Part model, mm, in its own coordinate system. Coordinates: 2 decimals unless noted, no trailing zeros. Loops run counter-clockwise (first coordinate to the right, second up) from the corner with the lowest first, then second, coordinate; pieces in that order, holes last. Notation, with made-up numbers: M -21.5,4 L 5.5,4 A33 cw 5.5,36 Z; hole C 88.25,-14 d3. An arc over 180 degrees is marked long. Answer as a JSON object with one key per item and string values. Group by question number.
1. Saw through at B-B on x = 9. Write the cut outline in (y, z).
2. Saw through at A-A on y = 26. Write the cut outline in (x, z) (3 decimals).
3. Drop flat-ended pins along their axis: pin 1 Ø10.5 at (y, z) = (26, -20) entering from +X; pin 2 Ø8.5 at (y, z) = (-27, 20) entering from -X; pin 3 Ø2.5 at (x, z) = (5, 30) entering from +Y. Give the stop position or say it passes through.
4. Drill centre lines: L1, parallel to Z at x = 4.75, y = 26; L2, parallel to Y at x = 3.75, z = -20; L3, parallel to X at y = 26.25, z = 30. Where is each one in solid material? Low to high.
5. Saw through at C-C on z = 20. Write the cut outline in (x, y) (3 decimals), then the cut area to 3 significant figures.
6. Saw through at D-D on y = -27. Write the cut outline in (x, z) (3 decimals).
from build123d import *

# Parameters (mm, degrees)
SKETCH_1_W                = 100
SKETCH_1_H                = 70
EXTRUDE_1_DEPTH           = 10
HOLE_WIZARD_1_D           = 6.6
HOLE_WIZARD_1_DEPTH       = 15
HOLE_WIZARD_1_CBORE_D     = 11
HOLE_WIZARD_1_CBORE_DEPTH = 6.8
HOLE_WIZARD_1_TIP         = 1.982840043
HOLE_WIZARD_3_AT_2_COUNT  = 2
HOLE_WIZARD_3_AT_2_PITCH  = 40
HOLE_WIZARD_3_AT_3_COUNT  = 2
HOLE_WIZARD_3_AT_3_PITCH  = 53
HOLE_WIZARD_3_AT_4_COUNT  = 2
HOLE_WIZARD_3_AT_4_PITCH  = 66.400301204
HOLE_WIZARD_M5_1_D        = 4.2
HOLE_WIZARD_M5_1_DEPTH    = 12.4
HOLE_WIZARD_M5_1_TIP      = 1.2618073


with BuildPart() as part:
    # 草图1 → 凸台-拉伸1 (new body)
    with BuildSketch(Plane(origin=(0, 0, 0), x_dir=(0, 0, -1), z_dir=(1, 0, 0))):
        Rectangle(SKETCH_1_W, SKETCH_1_H)
    extrude(amount=EXTRUDE_1_DEPTH)

    # 打孔尺寸(%根据)内六角圆柱头螺钉的类型1
    with Locations(Plane(origin=(10, 0, 0), x_dir=(0, 0, -1), z_dir=(1, 0, 0))):
        with Locations((-40, -5), (0, -5), (40, -5)):
            CounterBoreHole(HOLE_WIZARD_1_D / 2, HOLE_WIZARD_1_CBORE_D / 2, HOLE_WIZARD_1_CBORE_DEPTH, depth=HOLE_WIZARD_1_DEPTH)
            with Locations((0, 0, -(HOLE_WIZARD_1_DEPTH + HOLE_WIZARD_1_TIP / 2))):  # 118° drill point
                Cone(0, HOLE_WIZARD_1_D / 2, HOLE_WIZARD_1_TIP, mode=Mode.SUBTRACT)

    # 草图9 → 打孔尺寸(%根据)内六角圆柱头螺钉的类型3 (revolve, cut)
    with BuildSketch(Plane(origin=(0, 26, -20), x_dir=(0, 0, 1), z_dir=(0, 1, 0))):
        Polygon((0, 0), (0, 10), (3.3, 10), (3.3, 6.8), (5.5, 6.8), (5.5, 0.025), (5.525, 0), align=None)
    hole_wizard_3 = revolve(axis=Axis((-6.35, 26, -20), (1, 0, 0)), mode=Mode.SUBTRACT)

    # 打孔尺寸(%根据)内六角圆柱头螺钉的类型3 at 2: 打孔尺寸(%根据)内六角圆柱头螺钉的类型3 ×2
    with Locations(*[(0, 0, i * HOLE_WIZARD_3_AT_2_PITCH) for i in range(1, HOLE_WIZARD_3_AT_2_COUNT)]):
        add(hole_wizard_3, mode=Mode.SUBTRACT)

    # 打孔尺寸(%根据)内六角圆柱头螺钉的类型3 at 3: 打孔尺寸(%根据)内六角圆柱头螺钉的类型3 ×2
    with Locations(*[(0, -i * HOLE_WIZARD_3_AT_3_PITCH, 0) for i in range(1, HOLE_WIZARD_3_AT_3_COUNT)]):
        add(hole_wizard_3, mode=Mode.SUBTRACT)

    # 打孔尺寸(%根据)内六角圆柱头螺钉的类型3 at 4: 打孔尺寸(%根据)内六角圆柱头螺钉的类型3 ×2
    with Locations(*[Vector(0, -0.7981891503332307, 0.6024069059118724) * (i * HOLE_WIZARD_3_AT_4_PITCH) for i in range(1, HOLE_WIZARD_3_AT_4_COUNT)]):
        add(hole_wizard_3, mode=Mode.SUBTRACT)

    # M5 螺纹孔1
    with Locations(Plane(origin=(0, 35, 0), x_dir=(1, 0, 0), z_dir=(0, 1, 0))):
        with Locations((5, 30), (5, -30)):
            Hole(HOLE_WIZARD_M5_1_D / 2, depth=HOLE_WIZARD_M5_1_DEPTH)
            with Locations((0, 0, -(HOLE_WIZARD_M5_1_DEPTH + HOLE_WIZARD_M5_1_TIP / 2))):  # 118° drill point
                Cone(0, HOLE_WIZARD_M5_1_D / 2, HOLE_WIZARD_M5_1_TIP, mode=Mode.SUBTRACT)


solid = part.part
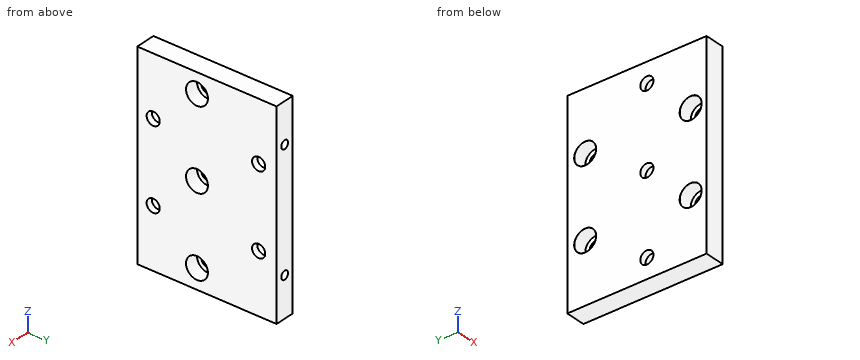
Outcome:
{
 "1": {"outline": "M -35,-50 L 35,-50 L 35,50 L -35,50 Z; hole C -27,-20 d6.6; hole C -27,20 d6.6; hole C -5,-40 d11; hole C -5,0 d11; hole C -5,40 d11; hole C 26,-20 d6.6; hole C 26,20 d6.6"},
 "2": {"outline": "M 0,-50 L 10,-50 L 10,-23.3 L 6.8,-23.3 L 6.8,-25.5 L 0.025,-25.5 L 0,-25.525 Z; M 0,-14.475 L 0.025,-14.5 L 6.8,-14.5 L 6.8,-16.7 L 10,-16.7 L 10,16.7 L 6.8,16.7 L 6.8,14.5 L 0.025,14.5 L 0,14.475 Z; M 0,25.525 L 0.025,25.5 L 6.8,25.5 L 6.8,23.3 L 10,23.3 L 10,50 L 0,50 Z; hole C 5,-30 d4.2; hole C 5,30 d4.2"},
 "3": {"pin 1": "stops at x = 10", "pin 2": "stops at x = 6.8", "pin 3": "stops at y = 22.09"},
 "4": {"L1": "z = -50 to -32.09, -27.91 to -25.5, -14.5 to 14.5, 25.5 to 27.91, 32.09 to 50", "L2": "y = -35 to -32.5, -21.5 to 20.5, 31.5 to 35", "L3": "x = 0 to 2.9, 7.1 to 10"},
 "5": {"outline": "M 0,-35 L 10,-35 L 10,-30.3 L 6.8,-30.3 L 6.8,-32.5 L 0.025,-32.5 L 0,-32.525 Z; M 0,-21.475 L 0.025,-21.5 L 6.8,-21.5 L 6.8,-23.7 L 10,-23.7 L 10,22.7 L 6.8,22.7 L 6.8,20.5 L 0.025,20.5 L 0,20.475 Z; M 0,31.525 L 0.025,31.5 L 6.8,31.5 L 6.8,29.3 L 10,29.3 L 10,35 L 0,35 Z", "area": "508 mm²"},
 "6": {"outline": "M 0,-50 L 10,-50 L 10,-23.3 L 6.8,-23.3 L 6.8,-25.5 L 0.025,-25.5 L 0,-25.525 Z; M 0,-14.475 L 0.025,-14.5 L 6.8,-14.5 L 6.8,-16.7 L 10,-16.7 L 10,16.7 L 6.8,16.7 L 6.8,14.5 L 0.025,14.5 L 0,14.475 Z; M 0,25.525 L 0.025,25.5 L 6.8,25.5 L 6.8,23.3 L 10,23.3 L 10,50 L 0,50 Z"}
}
